Can you work these out from the drawing? Everything is in mm from the part's minimum corner. A direction names the side the tool comes from. Round coordinates to 2 decimals unless told otherwise and drop trailing zeros. Loops run counter-clockwise (first coordinate to the right, second up) from the corner with the lowest first, then second, coordinate; pieces in that order, holes last. Notation, with made-up numbers: (76, -2.5) -> (109, -2.5) arc R34 cw to (109, 32.5) -> close; hole circle Ø11 at (39.25, 52.5). An arc over 180 degrees is marked (long way). Use CSV: the item, a comma, the result in double quotes. Start each with the question number.
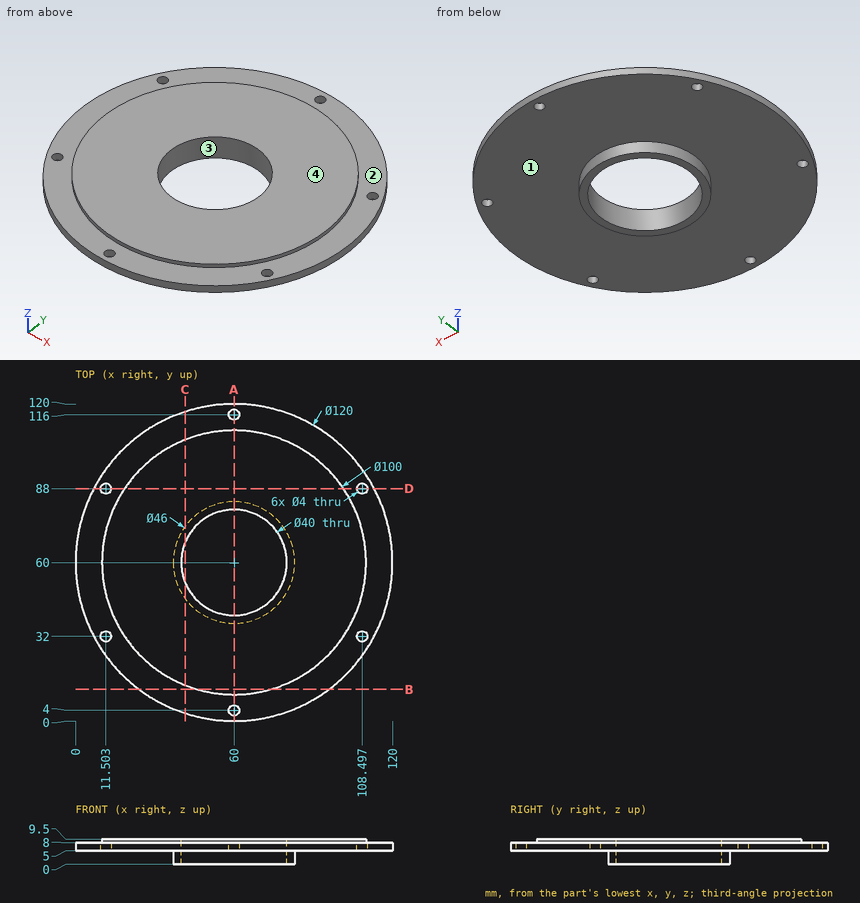
1. Suppose I cut it at B-B (y = 12). List the corners of the cut face in (x, z) for me, then the cut area to 3 significant figures.
2. Suppose I cut it at A-A (x = 60). List the corners of the cut face in (y, z) for me.
3. We'd pull the mould along X, two halves only. Please class the marked faces 3 and 4: pulls with the +X half, pulls with the -X half, needs draft (parallel to the pull), parting line crosses it, or undercut.
4. Suppose I cut it at D-D (y = 88). List the corners of the cut face in (x, z) for me (1 decimal).
5. For the marked faces 1 and 2, which set-ups out of +Z, -Z, +X, -X, +Y, -Y let a thin tool reach every point of the face, with its end or its side?
6. Will these pins go through, and if not, where does the flat tip stop? pin 1 (3 mm diameter, centred on x = 81.5, y = 34, fed in from -Z); pin 2 (4 mm diameter, centred on y = 37, z = 7, fed in from +X) (1 decimal); pin 3 (4 mm diameter, centred on x = 62.5, z = 3.5, fed in from -Y); pin 4 (3.5 mm diameter, centred on x = 108.5, y = 32, fed in from -Z).
7. Suppose I cut it at C-C (x = 41.5). List the corners of the cut face in (y, z) for me (1 decimal).
8. If I drill on L1, parallel to Y at x = 60, z = 7.3; L2, parallel to X at y = 60, z = 3; L3, parallel to X at y = 88, z = 6.35 (1 decimal), over which ranges is the centre line in solid material (lowest first)?
Geometry check:
1,outline,"(24, 5) -> (96, 5) -> (96, 8) -> (74, 8) -> (74, 9.5) -> (46, 9.5) -> (46, 8) -> (24, 8) -> close"
1,area,"258 mm²"
2,outline,"(0, 5) -> (2, 5) -> (2, 8) -> (0, 8) -> close; (6, 5) -> (37, 5) -> (37, 0) -> (40, 0) -> (40, 9.5) -> (10, 9.5) -> (10, 8) -> (6, 8) -> close; (80, 0) -> (83, 0) -> (83, 5) -> (114, 5) -> (114, 8) -> (110, 8) -> (110, 9.5) -> (80, 9.5) -> close; (118, 5) -> (120, 5) -> (120, 8) -> (118, 8) -> close"
3,face 3,"undercut"
3,face 4,"needs draft"
4,outline,"(6.9, 5) -> (9.5, 5) -> (9.5, 8) -> (6.9, 8) -> close; (13.5, 5) -> (106.5, 5) -> (106.5, 8) -> (101.4, 8) -> (101.4, 9.5) -> (18.6, 9.5) -> (18.6, 8) -> (13.5, 8) -> close; (110.5, 5) -> (113.1, 5) -> (113.1, 8) -> (110.5, 8) -> close"
5,face 1,"-Z"
5,face 2,"+Z"
6,pin 1,"stops at z = 5"
6,pin 2,"stops at x = 116.2"
6,pin 3,"stops at y = 0.01"
6,pin 4,"passes through"
7,outline,"(2.9, 5) -> (46.3, 5) -> (46.3, 0) -> (52.4, 0) -> (52.4, 9.5) -> (13.5, 9.5) -> (13.5, 8) -> (2.9, 8) -> close; (67.6, 0) -> (73.7, 0) -> (73.7, 5) -> (117.1, 5) -> (117.1, 8) -> (106.5, 8) -> (106.5, 9.5) -> (67.6, 9.5) -> close"
8,L1,"y = 0 to 2, 6 to 40, 80 to 114, 118 to 120"
8,L2,"x = 37 to 40, 80 to 83"
8,L3,"x = 6.9 to 9.5, 13.5 to 106.5, 110.5 to 113.1"
